```python
from build123d import *

# Parameters (mm, degrees)
BOSS_EXTRUDE1_DEPTH        = 10
M36X2_0_TAPPED_HOLE1_D     = 34
M36X2_0_TAPPED_HOLE1_DEPTH = 82
M36X2_0_TAPPED_HOLE1_TIP   = 10.214630523
SKETCH4_W                  = 19.309531336
SKETCH4_H                  = 7.869851007
CUT_EXTRUDE1_DEPTH         = 88
CIRPATTERN1_COUNT          = 6


with BuildPart() as part:
    # Sketch1 → Boss-Extrude1 (new body)
    with BuildSketch(Plane(origin=(0, 0, 0), x_dir=(1, 0, 0), z_dir=(0, 1, 0))):
        Polygon((22.5, -12.990381057), (22.5, 12.990381057), (0, 25.980762114), (-22.5, 12.990381057), (-22.5, -12.990381057), (0, -25.980762114), align=None)
    extrude(amount=BOSS_EXTRUDE1_DEPTH)

    # M36x2.0 Tapped Hole1
    with Locations(Plane(origin=(0, 10, 0), x_dir=(1, 0, 0), z_dir=(0, 1, 0))):
        with Locations((0, 0)):
            Hole(M36X2_0_TAPPED_HOLE1_D / 2, depth=M36X2_0_TAPPED_HOLE1_DEPTH)
            with Locations((0, 0, -(M36X2_0_TAPPED_HOLE1_DEPTH + M36X2_0_TAPPED_HOLE1_TIP / 2))):  # 118° drill point
                Cone(0, M36X2_0_TAPPED_HOLE1_D / 2, M36X2_0_TAPPED_HOLE1_TIP, mode=Mode.SUBTRACT)

    # Sketch4 → Cut-Extrude1 (cut)
    with BuildSketch(Plane(origin=(0, 10, 0), x_dir=(1, 0, 0), z_dir=(0, 1, 0))):
        with Locations((1.413316262, 28.934925504)):
            Rectangle(SKETCH4_W, SKETCH4_H)
    cut_extrude1 = extrude(amount=-CUT_EXTRUDE1_DEPTH, mode=Mode.SUBTRACT)

    # CirPattern1: Cut-Extrude1 ×6 about axis
    cirpattern1_axis = Axis((0, 0, 0), (0, 1, 0))
    for i in range(1, CIRPATTERN1_COUNT):
        add(cut_extrude1.rotate(cirpattern1_axis, i * 360 / CIRPATTERN1_COUNT), mode=Mode.SUBTRACT)


solid = part.part
```
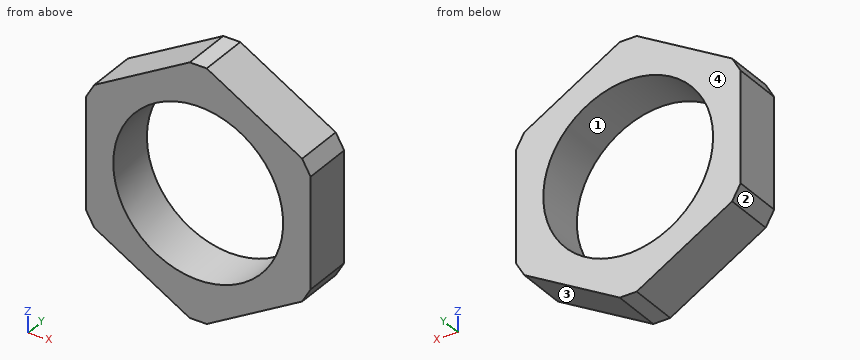
The listing builds one solid part. Answer for the finished solid, in the listing's coordinates (mm). Face numbers are marked on the shaded views. Round coordinates to 2 decimals unless told otherwise and drop trailing zeros. Loops run counter-clockwise (first coordinate to the right, second up) from the corner with the lowest first, then second, coordinate; pieces in that order, holes last. Notation, with made-up numbers: (64.5, -34.75) - (100.5, -34.75) arc R15 cw to (100.5, -30.75) - close; hole circle Ø11 at (23.5, 10). An arc over 180 degrees is marked (long way). Return JSON: item names as keys, results as strings. Group by question number.
1. The part is cut by section D-D on z = -20. Determine the outline of the cut face in (x, y), then the cut area to 3 significant figures.
2. The mould has two halves that part along X. Classify the marked faces 1, 2, 3 and 4: pulls with the +X half, pulls with the -X half, needs draft (parallel to the pull), parting line crosses it, or undercut.
3. The part is cut by section A-A on z = -8. Determine the outline of the cut face in (x, y).
4. Consider probe 1 along Z at (x, y) = (0, 4.75); probe 2 along X at (y, z) = (0.5, 15); probe 3 along Z at (x, y) = (6.5, 6). Determine where each line is inside the solid, lowest interval first.
5. The part is cut by section C-C on y = 4.75. Determine the outline of the cut face in (x, z).
6. The part is cut by section B-B on x = 0. Determine the outline of the cut face in (y, z), then the cut area to 3 significant figures.
7. Each of these flat-tipped pins is pushed along its axis until it touches: P1, Ø4, axis at x = -10, z = 11, coming from the -Y side; P2, Ø3, axis at x = 9, y = 4, coming from the +Z side; P3, Ø2, axis at y = 1, z = 14, coming from the -X side; P4, Ø3, axis at x = -5.5, y = 6, coming from the -Z side. Where does it stop, or does it pass through?
Resolved:
{
 "1": {"outline": "(-10.36, 0) - (10.36, 0) - (10.36, 10) - (-10.36, 10) - close", "area": "207 mm²"},
 "2": {"face 1": "undercut", "face 2": "pulls with the -X half", "face 3": "pulls with the +X half", "face 4": "needs draft"},
 "3": {"outline": "(-22.5, 0) - (-15, 0) - (-15, 10) - (-22.5, 10) - close; (15, 0) - (22.5, 0) - (22.5, 10) - (15, 10) - close"},
 "4": {"probe 1": "z = -25 to -17, 17 to 25", "probe 2": "x = -19.02 to -8, 8 to 19.02", "probe 3": "z = -22.23 to -15.71, 15.71 to 22.23"},
 "5": {"outline": "(-22.5, -11.03) - (-20.8, -13.97) - (-1.7, -25) - (1.7, -25) - (20.8, -13.97) - (22.5, -11.03) - (22.5, 11.03) - (20.8, 13.97) - (1.7, 25) - (-1.7, 25) - (-20.8, 13.97) - (-22.5, 11.03) - close; hole circle Ø34 at (0, 0)"},
 "6": {"outline": "(0, -25) - (10, -25) - (10, -17) - (0, -17) - close; (0, 17) - (10, 17) - (10, 25) - (0, 25) - close", "area": "160 mm²"},
 "7": {"P1": "passes through", "P2": "stops at z = 21.65", "P3": "stops at x = -21.36", "P4": "stops at z = -23.67"}
}
